from build123d import *

# Parameters (mm, degrees)
SKETCH1_R             = 3
BOSS_EXTRUDE1_DEPTH   = 60
M4_TAPPED_HOLE1_D     = 3.3
M4_TAPPED_HOLE1_DEPTH = 10.1
M4_TAPPED_HOLE1_TIP   = 0.991420021
M4_TAPPED_HOLE2_D     = 3.3
M4_TAPPED_HOLE2_DEPTH = 10.1
M4_TAPPED_HOLE2_TIP   = 0.991420021


with BuildPart() as part:
    # Sketch1 → Boss-Extrude1 (new, symmetric)
    with BuildSketch(Plane.XY):
        Circle(SKETCH1_R)
    extrude(amount=BOSS_EXTRUDE1_DEPTH, both=True)

    # M4 Tapped Hole1
    with Locations(Plane.XY.offset(60)):
        with Locations((0, 0)):
            Hole(M4_TAPPED_HOLE1_D / 2, depth=M4_TAPPED_HOLE1_DEPTH)
            with Locations((0, 0, -(M4_TAPPED_HOLE1_DEPTH + M4_TAPPED_HOLE1_TIP / 2))):  # 118° drill point
                Cone(0, M4_TAPPED_HOLE1_D / 2, M4_TAPPED_HOLE1_TIP, mode=Mode.SUBTRACT)

    # M4 Tapped Hole2
    with Locations(Plane(origin=(0, 0, -60), x_dir=(-1, 0, 0), z_dir=(0, 0, -1))):
        with Locations((0, 0)):
            Hole(M4_TAPPED_HOLE2_D / 2, depth=M4_TAPPED_HOLE2_DEPTH)
            with Locations((0, 0, -(M4_TAPPED_HOLE2_DEPTH + M4_TAPPED_HOLE2_TIP / 2))):  # 118° drill point
                Cone(0, M4_TAPPED_HOLE2_D / 2, M4_TAPPED_HOLE2_TIP, mode=Mode.SUBTRACT)


solid = part.part
The listing builds one solid part. Answer for the finished solid, in the listing's coordinates (mm). A direction names the side the tool comes from. Give positions to 0.01 mm unless a question says otherwise; leave off trailing zeros. Write each loop counter-clockwise with the first axis right and the second up, starting at its lowest first coordinate (ties: lowest second). Pieces come first, ordered by that corner, then holes.
1) For a pull along Y with two mould halves and no side action, classify faces 4 (the face through (1.3, -1.3, -60)), 5 (the face through (-3, 0, 1)), 6 (the face through (-0.1, -0.3, 49.1)) as pulls with the +Y half, pulls with the -Y half, needs draft (parallel to the pull), parting line crosses it, or undercut.
2) Section A-A (z = 41) is taken. Write down the section's boundary in (x, y).
3) A tool of negligible diameter and unlimited length cuts with its end or side. For faces 1 (the face through (-1.216, 1.115, -54.879)), 2 (the face through (1.216, 1.115, 54.879)), 3 (the face through (1.3, -1.3, 60)), from which of +Z, -Z, +X, -X, +Y, -Y can it reach the whole face along a straight path? Write none if from no direction.
4) Given P1, Ø1.5, axis at x = 1, z = 38, coming from the +Y side; P2, Ø2.5, axis at x = 0, y = 0, coming from the -Z side, each flat-ended and moving along its own axis, determine where each tip first touches the part or whether it passes through.
5) Find the intervals of material crossed by L1, parallel to Y at x = 0, z = -56; L2, parallel to X at y = 0.2, z = 30; L3, parallel to X at y = -0.45, z = -53.5, in increasing order.
Response:
1. face 4: needs draft
1. face 5: parting line crosses it
1. face 6: undercut
2. outline: circle Ø6 at (0, 0)
3. face 1: -Z
3. face 2: +Z
3. face 3: +Z, +X, -X, +Y, -Y
4. P1: stops at y = 2.99
4. P2: stops at z = -49.66
5. L1: y = -3 to -1.65, 1.65 to 3
5. L2: x = -2.99 to 2.99
5. L3: x = -2.97 to -1.59, 1.59 to 2.97
